For this review, take the finished solid that the model builds, in its own axes (mm). Coordinates: 2 decimals unless noted, no trailing zeros. Write each loop counter-clockwise with the first axis right and the second up, starting at its lowest first coordinate (ties: lowest second). Pieces come first, ordered by that corner, then holes. Notation, with made-up numbers: M 5.5,53.5 L 61.5,53.5 A17 cw 61.5,59.5 Z; hole C 82.25,36.5 d3. An arc over 180 degrees is marked long. One line per question, with ' | ' between items.
from build123d import *

# Parameters (mm, degrees)
SKETCH1_R           = 47.25
SKETCH1_R_2         = 10.1
BOSS_EXTRUDE1_DEPTH = 1
BOSS_EXTRUDE2_DEPTH = 1
CUT_EXTRUDE1_DEPTH  = 10


with BuildPart() as part:
    # Sketch1 → Boss-Extrude1 (new body)
    with BuildSketch(Plane(origin=(0, 0, 0), x_dir=(1, 0, 0), z_dir=(0, 1, 0))):
        with Locations(Location((0, 0, 0), (0, 0, 270))):
            Circle(SKETCH1_R)
        with Locations(Location((0, 0, 0), (0, 0, 270))):
            Circle(SKETCH1_R_2, mode=Mode.SUBTRACT)
    extrude(amount=BOSS_EXTRUDE1_DEPTH)

    # Sketch2 → Boss-Extrude2 (add)
    with BuildSketch(Plane.XZ):
        with BuildLine():
            Line((6.033241252, -8.1), (-6.033241252, -8.1))
            ThreePointArc((-6.033241252, -8.1), (0, -10.1), (6.033241252, -8.1))
        make_face()
        with BuildLine():
            Line((6.033241252, 8.1), (-6.033241252, 8.1))
            ThreePointArc((-6.033241252, 8.1), (0, 10.1), (6.033241252, 8.1))
        make_face()
    extrude(amount=-BOSS_EXTRUDE2_DEPTH)

    # Sketch3 → Cut-Extrude1 (cut)
    with BuildSketch(Plane.XZ):
        with BuildLine():
            Line((0, 47.25), (0, 36.5))
            ThreePointArc((0, 36.5), (-36.5, 0), (0, -36.5))
            Line((0, -36.5), (0, -47.25))
            ThreePointArc((0, -47.25), (-47.25, 0), (0, 47.25))
        make_face()
    extrude(amount=-CUT_EXTRUDE1_DEPTH, mode=Mode.SUBTRACT)


solid = part.part
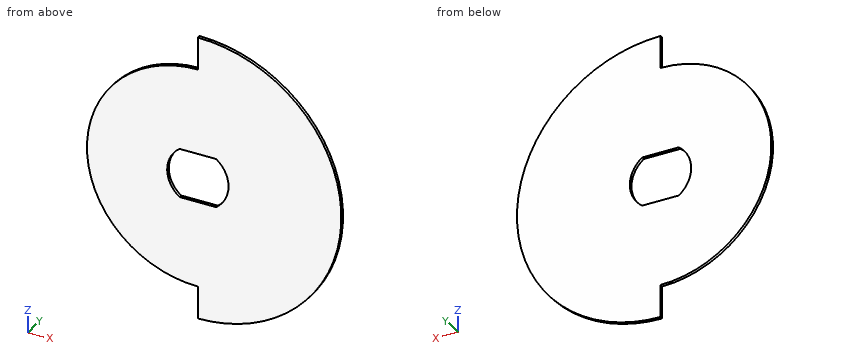
1. Take a section at C-C on x = 3. State the section outline as (y, z) points, plus the area to 3 significant figures.
Computed values:
outline: M 0,-47.15 L 1,-47.15 L 1,-8.1 L 0,-8.1 Z; M 0,8.1 L 1,8.1 L 1,47.15 L 0,47.15 Z | area: 78.1 mm2
2. Take a section at B-B on y = 0.25. State the section outline as (x, z) points, plus the area to 3 significant figures.
Computed values:
outline: M 0,-47.25 A47.25 ccw 0,47.25 L 0,36.5 A36.5 ccw 0,-36.5 Z; hole M -6.03,-8.1 L 6.03,-8.1 A10.1 ccw 6.03,8.1 L -6.03,8.1 A10.1 ccw Z | area: 5,310 mm2
3. Take a section at D-D on z = 10. State the section outline as (x, y) points, plus the area to 3 significant figures.
Computed values:
outline: M -35.1,0 L 46.18,0 L 46.18,1 L -35.1,1 Z | area: 81.3 mm2
4. Take a section at A-A on z = 0. State the section outline as (x, y) points.
Computed values:
outline: M -36.5,0 L -10.1,0 L -10.1,1 L -36.5,1 Z; M 10.1,0 L 47.25,0 L 47.25,1 L 10.1,1 Z
5. For line 1 along Z through (x, y) = (-0.5, 0.8); line 2 along X through (y, z) = (0.4, 0); line 3 along X through (y, z) = (0.55, -7.5), list the stretches that pass through material, from the lowest coordinate up.
Computed values:
line 1: z = -36.5 to -8.1, 8.1 to 36.5 | line 2: x = -36.5 to -10.1, 10.1 to 47.25 | line 3: x = -35.72 to -6.76, 6.76 to 46.65
